Read the model definition and answer for the solid it produces. Units are mm, in the model's axes. A direction names the side the tool comes from. Round coordinates to 2 decimals unless told otherwise and drop trailing zeros. Order: outer loops, then holes, each group sorted by start corner. A loop starts at its lowest first (then second) coordinate and runs counter-clockwise, first axis right, second up. Notation, with made-up numbers: (86.5, -25.5) - (124.5, -25.5) arc R20 cw to (124.5, -19.5) - close; hole circle Ø11 at (13.5, 22). An arc over 180 degrees is marked (long way). Answer as a JSON object with one key per item and string values. Group by question number.
Q1. Consider line 1 (X direction, y = -64.5, z = -13.5); line 2 (X direction, y = -1, z = 11); line 3 (Z direction, x = -3.5, y = 22). Determine where each line is inside the solid, lowest interval first.
Q2. A cutting plane is placed at B-B on x = 0. Determine the outline of the cut face in (y, z), and give its area (3 significant figures).
Q3. Given pin 1 Ø15 at (y, z) = (-52.5, -5.5) entering from +X; pin 2 Ø2 at (x, z) = (-18, 3) entering from -Y; pin 3 Ø1.5 at (x, z) = (10.5, -11) entering from +Y; pin 4 Ø15.5 at (y, z) = (-60, 0) entering from +X, each flat-ended and moving along its own axis, determine where each tip first touches the part or whether it passes through.
Q4. A cutting plane is placed at D-D on z = -10. Determine the outline of the cut face in (x, y).
Q5. A tool of negligible diameter and unlimited length cuts with its end or side. For faces 1 (the cylindrical face through (-0.7, 22.49, 9.08)), 2 (the cylindrical face through (0.501, 17.493, -9.084)), 3 (the flat face through (-10, -37, 0)), 4 (the flat face through (15, -43, 0)), from which of +Z, -Z, +X, -X, +Y, -Y can it reach the whole face along a straight path? Write none if from no direction.
Q6. A cutting plane is placed at C-C on z = 5. Determine the outline of the cut face in (x, y), and give its area (3 significant figures).
Q7. The mould has two halves that part along Z. Classify faces 5 (the cylindrical face through (-12.465, -51.776, 2.59)), 6 (the flat face through (0, 18, -3)), 7 (the flat face through (-15, -44, 0)): pulls with the +Z half, pulls with the -Z half, needs draft (parallel to the pull), parting line crosses it, or undercut.
Q8. A cutting plane is placed at A-A on y = -39. Determine the outline of the cut face in (x, z), and give its area (3 significant figures).
```python
from build123d import *

# Parameters (mm, degrees)
CLEVIS_BODY_DEPTH        = 15
PROFILE_START            = 15
PROFILE_CUT_A_12MM_DEPTH = 12
PROFILE_START_2          = -15
PROFILE_CUT_B_12MM_DEPTH = 12
HEAD_SLOT_SKETCH_R       = 8.62165443
HEAD_SLOT_CUT_DEPTH      = 88.5


with BuildPart() as part:
    # Clevis Profile Sketch → Clevis Body (new, symmetric)
    # profile 1 of 3: a face of its own
    with BuildSketch(Plane.XY):
        with BuildLine():
            ThreePointArc((-15, 0), (0, 15), (15, 0))
            Line((15, 0), (15, -23.048861143))
            ThreePointArc((15, -23.048861143), (0, 27.5), (-15, -23.048861143))
            Line((-15, -23.048861143), (-15, 0))
        make_face()
        with BuildLine():
            ThreePointArc((-17.692907365, -13.900037013), (0, 22.5), (17.692907365, -13.900037013))
            ThreePointArc((17.692907365, -13.900037013), (15.892818017, -11.22254507), (15.557337138, -8.013692106))
            ThreePointArc((15.557337138, -8.013692106), (0, 17.5), (-15.557337138, -8.013692106))
            ThreePointArc((-15.557337138, -8.013692106), (-15.892818017, -11.22254507), (-17.692907365, -13.900037013))
        make_face(mode=Mode.SUBTRACT)
    # profile 2 of 3: a face of its own
    with BuildSketch(Plane.XY):
        with BuildLine():
            ThreePointArc((17.692907365, -13.900037013), (15.892818017, -11.22254507), (15.557337138, -8.013692106))
            ThreePointArc((15.557337138, -8.013692106), (0, 17.5), (-15.557337138, -8.013692106))
            ThreePointArc((-15.557337138, -8.013692106), (-15.892818017, -11.22254507), (-17.692907365, -13.900037013))
            ThreePointArc((-17.692907365, -13.900037013), (0, 22.5), (17.692907365, -13.900037013))
        make_face()
    # profile 3 of 3: a face of its own
    with BuildSketch(Plane.XY):
        with BuildLine():
            ThreePointArc((10, 0), (0, 10), (-10, 0))
            Line((-10, 0), (-10, -75))
            Line((-10, -75), (-15, -75))
            Line((-15, -75), (-15, 0))
            ThreePointArc((-15, 0), (0, 15), (15, 0))
            Line((15, 0), (15, -75))
            Line((15, -75), (10, -75))
            Line((10, -75), (10, 0))
        make_face()
    extrude(amount=CLEVIS_BODY_DEPTH, both=True)

    # Sketch1_3 → Profile Cut A 12mm (cut)
    with BuildSketch(Plane.XY.offset(PROFILE_START)):
        with BuildLine():
            ThreePointArc((17.692907365, -13.900037013), (15.892818017, -11.22254507), (15.557337138, -8.013692106))
            ThreePointArc((15.557337138, -8.013692106), (0, 17.5), (-15.557337138, -8.013692106))
            ThreePointArc((-15.557337138, -8.013692106), (-15.892818017, -11.22254507), (-17.692907365, -13.900037013))
            ThreePointArc((-17.692907365, -13.900037013), (0, 22.5), (17.692907365, -13.900037013))
        make_face()
    extrude(amount=-PROFILE_CUT_A_12MM_DEPTH, mode=Mode.SUBTRACT)

    # Sketch1_4 → Profile Cut B 12mm (cut)
    with BuildSketch(Plane.XY.offset(PROFILE_START_2)):
        with BuildLine():
            ThreePointArc((17.692907365, -13.900037013), (15.892818017, -11.22254507), (15.557337138, -8.013692106))
            ThreePointArc((15.557337138, -8.013692106), (0, 17.5), (-15.557337138, -8.013692106))
            ThreePointArc((-15.557337138, -8.013692106), (-15.892818017, -11.22254507), (-17.692907365, -13.900037013))
            ThreePointArc((-17.692907365, -13.900037013), (0, 22.5), (17.692907365, -13.900037013))
        make_face()
    extrude(amount=PROFILE_CUT_B_12MM_DEPTH, mode=Mode.SUBTRACT)

    # Head Slot Sketch → Head Slot Cut (cut, through all)
    with BuildSketch(Plane(origin=(15, 0, 0), x_dir=(0, 0, -1), z_dir=(1, 0, 0))):
        with Locations(Location((0, -59.999173584, 0), (0, 0, 90))):
            Circle(HEAD_SLOT_SKETCH_R)
        with BuildLine():
            Line((-15, -75), (0, -75))
            ThreePointArc((0, -75), (-10.55136927, -70.661884294), (-15, -60.15663199))
            Line((-15, -60.15663199), (-15, -75))
        make_face()
        with BuildLine():
            Line((15, -75), (15, -60.15663199))
            ThreePointArc((15, -60.15663199), (10.55136927, -70.661884294), (0, -75))
            Line((0, -75), (15, -75))
        make_face()
    extrude(amount=-HEAD_SLOT_CUT_DEPTH, mode=Mode.SUBTRACT)


solid = part.part
```
Result set:
{
 "1": {"line 1": "x = -15 to -10, 10 to 15", "line 2": "x = -27.48 to -22.48, -17.47 to -10, 10 to 17.47, 22.48 to 27.48", "line 3": "z = -3 to 3"},
 "2": {"outline": "(10, -15) - (17.5, -15) - (17.5, -3) - (22.5, -3) - (22.5, -15) - (27.5, -15) - (27.5, 15) - (22.5, 15) - (22.5, 3) - (17.5, 3) - (17.5, 15) - (10, 15) - close", "area": "405 mm²"},
 "3": {"pin 1": "stops at x = 15", "pin 2": "stops at y = -21.62", "pin 3": "stops at y = 25.71", "pin 4": "passes through"},
 "4": {"outline": "(-15, -71.18) - (-10, -71.18) - (-10, 0) arc R10 cw to (10, 0) - (10, -71.18) - (15, -71.18) - (15, -23.05) arc R27.5 ccw (long way) to (-15, -23.05) - close; hole (-17.69, -13.9) arc R6.68 ccw to (-15.56, -8.01) arc R17.5 cw (long way) to (15.56, -8.01) arc R6.68 ccw to (17.69, -13.9) arc R22.5 ccw (long way) to start"},
 "5": {"face 1": "+Z", "face 2": "-Z", "face 3": "+Z, -Z, -Y", "face 4": "+Z, -Z, +X, -Y"},
 "6": {"outline": "(-15, -74.14) - (-10, -74.14) - (-10, -67.02) - (-15, -67.02) - close; (-15, -52.98) - (-10, -52.98) - (-10, 0) arc R10 cw to (10, 0) - (10, -52.98) - (15, -52.98) - (15, -23.05) arc R27.5 ccw (long way) to (-15, -23.05) - close; (10, -74.14) - (15, -74.14) - (15, -67.02) - (10, -67.02) - close; hole (-17.69, -13.9) arc R6.68 ccw to (-15.56, -8.01) arc R17.5 cw (long way) to (15.56, -8.01) arc R6.68 ccw to (17.69, -13.9) arc R22.5 ccw (long way) to start", "area": "1,600 mm²"},
 "7": {"face 5": "undercut", "face 6": "pulls with the -Z half", "face 7": "needs draft"},
 "8": {"outline": "(-15, -15) - (-10, -15) - (-10, 15) - (-15, 15) - close; (10, -15) - (15, -15) - (15, 15) - (10, 15) - close", "area": "300 mm²"}
}
